from build123d import *

# Parameters (mm, degrees)
EXTRUDE1_DEPTH         = 1124
SKETCH2_W              = 32
SKETCH2_H              = 32
CUT_EXTRUDE1_DEPTH     = 1128.553102962
SKETCH3_W              = 32
SKETCH3_H              = 4
CUT_EXTRUDE2_DEPTH     = 1200
CUT_EXTRUDE3_DEPTH     = 1128.553102962
LPATTERN1_COUNT        = 4
LPATTERN1_PITCH        = 40
LPATTERN2_COUNT        = 2
LPATTERN2_PITCH        = 350
LPATTERN2_COPY_1_DEPTH = 1128.553102962
LPATTERN2_COPY_2_DEPTH = 1128.553102962
LPATTERN2_COPY_3_DEPTH = 1128.553102962


with BuildPart() as part:
    # Sketch1 → Extrude1 (new body)
    with BuildSketch(Plane.XY):
        Polygon((0, 0), (-40, 0), (-40, 80), (0, 80), (0, 76), (-32, 76), (-32, 4), (0, 4), align=None)
    extrude(amount=EXTRUDE1_DEPTH)

    # Sketch2 → Cut-Extrude1 (cut, through all)
    with BuildSketch(Plane(origin=(0, 80, 0), x_dir=(1, 0, 0), z_dir=(0, 1, 0))):
        with Locations((-16, -16)):
            Rectangle(SKETCH2_W, SKETCH2_H)
        with Locations((-16, -1108)):
            Rectangle(SKETCH2_W, SKETCH2_H)
    extrude(amount=-CUT_EXTRUDE1_DEPTH, mode=Mode.SUBTRACT)

    # Sketch3 → Cut-Extrude2 (cut)
    with BuildSketch(Plane(origin=(-32, 0, 0), x_dir=(0, 0, -1), z_dir=(1, 0, 0))):
        with Locations((-1108, 78)):
            Rectangle(SKETCH3_W, SKETCH3_H)
        with Locations((-1108, 2)):
            Rectangle(SKETCH3_W, SKETCH3_H)
        with Locations((-16, 78)):
            Rectangle(SKETCH3_W, SKETCH3_H)
        with Locations((-16, 2)):
            Rectangle(SKETCH3_W, SKETCH3_H)
    extrude(amount=-CUT_EXTRUDE2_DEPTH, mode=Mode.SUBTRACT)

    # Sketch4 → Cut-Extrude3 (cut, through all)
    with BuildSketch(Plane(origin=(0, 80, 0), x_dir=(1, 0, 0), z_dir=(0, 1, 0))):
        with BuildLine():
            Line((-29.5, -924), (-29.5, -940))
            ThreePointArc((-29.5, -940), (-22.5, -947), (-15.5, -940))
            Line((-15.5, -940), (-15.5, -924))
            ThreePointArc((-15.5, -924), (-22.5, -917), (-29.5, -924))
        make_face()
    cut_extrude3 = extrude(amount=-CUT_EXTRUDE3_DEPTH, mode=Mode.SUBTRACT)

    # LPattern1: Cut-Extrude3 ×4
    with Locations(*[(0, 0, -i * LPATTERN1_PITCH) for i in range(1, LPATTERN1_COUNT)]):
        add(cut_extrude3, mode=Mode.SUBTRACT)

    # LPattern2: Cut-Extrude3 ×2
    with Locations(*[(0, 0, -i * LPATTERN2_PITCH) for i in range(1, LPATTERN2_COUNT)]):
        add(cut_extrude3, mode=Mode.SUBTRACT)

    # LPattern2 copy 1 sketch → LPattern2 copy 1 (cut, through all)
    with BuildSketch(Plane(origin=(0, 80, -390), x_dir=(1, 0, 0), z_dir=(0, 1, 0))):
        with BuildLine():
            Line((-29.5, -924), (-29.5, -940))
            ThreePointArc((-29.5, -940), (-22.5, -947), (-15.5, -940))
            Line((-15.5, -940), (-15.5, -924))
            ThreePointArc((-15.5, -924), (-22.5, -917), (-29.5, -924))
        make_face()
    extrude(amount=-LPATTERN2_COPY_1_DEPTH, mode=Mode.SUBTRACT)

    # LPattern2 copy 2 sketch → LPattern2 copy 2 (cut, through all)
    with BuildSketch(Plane(origin=(0, 80, -430), x_dir=(1, 0, 0), z_dir=(0, 1, 0))):
        with BuildLine():
            Line((-29.5, -924), (-29.5, -940))
            ThreePointArc((-29.5, -940), (-22.5, -947), (-15.5, -940))
            Line((-15.5, -940), (-15.5, -924))
            ThreePointArc((-15.5, -924), (-22.5, -917), (-29.5, -924))
        make_face()
    extrude(amount=-LPATTERN2_COPY_2_DEPTH, mode=Mode.SUBTRACT)

    # LPattern2 copy 3 sketch → LPattern2 copy 3 (cut, through all)
    with BuildSketch(Plane(origin=(0, 80, -470), x_dir=(1, 0, 0), z_dir=(0, 1, 0))):
        with BuildLine():
            Line((-29.5, -924), (-29.5, -940))
            ThreePointArc((-29.5, -940), (-22.5, -947), (-15.5, -940))
            Line((-15.5, -940), (-15.5, -924))
            ThreePointArc((-15.5, -924), (-22.5, -917), (-29.5, -924))
        make_face()
    extrude(amount=-LPATTERN2_COPY_3_DEPTH, mode=Mode.SUBTRACT)


solid = part.part
The listing builds one solid part. Answer for the finished solid, in the listing's coordinates (mm). A direction names the side the tool comes from. Round coordinates to 2 decimals unless told otherwise and drop trailing zeros. Order: outer loops, then holes, each group sorted by start corner. A loop starts at its lowest first (then second) coordinate and runs counter-clockwise, first axis right, second up. Notation, with made-up numbers: (81, -7) - (91, -7) arc R33 ccw to (91, 22) - close; hole circle Ø4 at (-25.75, 79). An arc over 180 degrees is marked (long way). Write item = value, one per line. Start each with the question number.
1) Section C-C, the plane y = 66.5 is taken. Write down the section's boundary in (x, z), plus the area to 3 significant figures.
2) Straight lines are drawn through the part: L1, parallel to Y at x = -27, z = 788; L2, parallel to X at y = 26, z = 854.5. For each, find the intervals that lie inside material, in ascending order.
3) Section A-A, the plane z = 404 is taken. Write down the section's boundary in (x, y).
4) Section B-B, the plane x = -22.5 is taken. Count the separate pieces of the cut face and the enclosed holes in it, plus the area to 3 significant figures.
5) For faces 4 (the flat face through (-32, 41, 570)), 5 (the flat face through (-40, 39, 554)), determine the directions among +Z, -Z, +X, -X, +Y, -Y from which every point of the face is accessible in a straight line to the end or side of a thin tool.
6) For a pull along Y with two mould halves and no side action, classify faces 1 (the flat face through (-16, 76, 555)), 2 (the flat face through (-16, 80, 555)), 3 (the flat face through (-15, 0, 555)) as released by +Y, released by -Y, zero draft, split by the parting line, or undercut.
7) Given pin 1 (4 mm diameter, centred on y = 50, z = 418, fed in from +X); pin 2 (6.5 mm diameter, centred on x = -36.5, z = 1107.5, fed in from -Y), each flat-ended and moving along its own axis, determine where each tip first touches the part or whether it passes through.
Results list:
q1.outline = (-40, 0) - (-32, 0) - (-32, 1124) - (-40, 1124) - close
q1.area = 8,990 mm^2
q2.L1 = 0 to 4, 76 to 80
q2.L2 = -40 to -32
q3.outline = (-40, 0) - (0, 0) - (0, 4) - (-32, 4) - (-32, 76) - (0, 76) - (0, 80) - (-40, 80) - close
q4.separate_pieces = 18
q4.enclosed_holes = 0
q4.area = 6,560 mm^2
q5.face_4 = +Z, -Z, +X
q5.face_5 = +Z, -Z, -X, +Y, -Y
q6.face_1 = undercut
q6.face_2 = released by +Y
q6.face_3 = released by -Y
q7.pin_1 = -32
q7.pin_2 = 4
